Design review of the part shown in the three views and the two pictorial views. Dimensions are in mm from the part's minimum x, y and z. A direction names the side the tool comes from. Coordinates: 2 decimals unless noted, no trailing zeros. Loops run counter-clockwise (first coordinate to the right, second up) from the corner with the lowest first, then second, coordinate; pieces in that order, holes last. Notation, with made-up numbers: (44.25, -26) -> (82.25, -26) arc R6 cw to (82.25, -20) -> close; hole circle Ø8 at (9, 51.25). An arc over 180 degrees is marked (long way). Use CSV: the item, a comma, the result in double quotes.
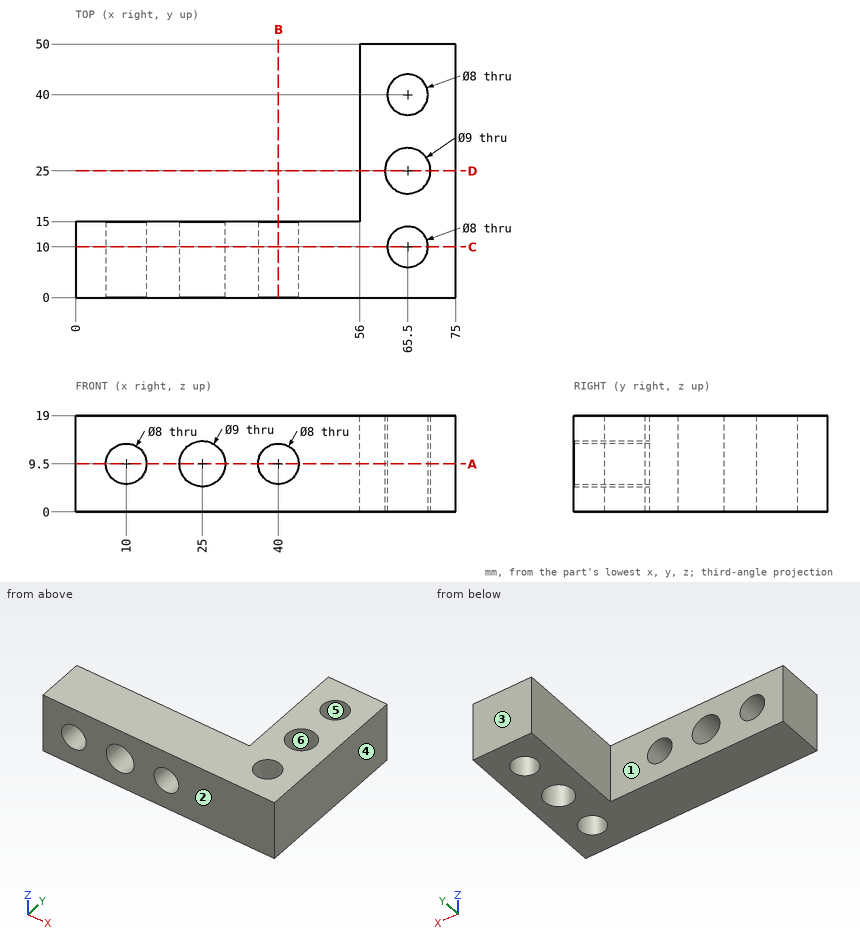
Item 1: Add section D-D (y = 25). Give the boundary of the cut face in (x, z), then the cut area to 3 significant figures.
Checked values:
outline,"(56, 0) -> (61, 0) -> (61, 19) -> (56, 19) -> close; (70, 0) -> (75, 0) -> (75, 19) -> (70, 19) -> close"
area,"190 mm^2"
Item 2: Machinability: for the marked faces 1 and 2, which of the approach directions +Z, -Z, +X, -X, +Y, -Y give a long, thin tool a straight path to every point of the face, cutting with its end or side? Answer none if there is none.
Checked values:
face 1,"+Z, -Z, -X, +Y"
face 2,"+Z, -Z, +X, -X, -Y"
Item 3: Add section C-C (y = 10). Give the boundary of the cut face in (x, z).
Checked values:
outline,"(0, 0) -> (61.5, 0) -> (61.5, 19) -> (0, 19) -> close; (69.5, 0) -> (75, 0) -> (75, 19) -> (69.5, 19) -> close; hole circle Ø8 at (10, 9.5); hole circle Ø9 at (25, 9.5); hole circle Ø8 at (40, 9.5)"
Item 4: Draft analysis for pull direction Y (two halves, no side actions). For the marked faces 3, 4, 5 and 6, state which applies: pulls with the +Y half, pulls with the -Y half, needs draft (parallel to the pull), parting line crosses it, or undercut.
Checked values:
face 3,"pulls with the +Y half"
face 4,"needs draft"
face 5,"undercut"
face 6,"undercut"
Item 5: Clearance check with flat-ended pins moving along their axes: pin 1 (7 mm diameter, centred on x = 65.5, y = 25, fed in from -Z); pin 2 (5.5 mm diameter, centred on y = 39, z = 5, fed in from -X); pin 3 (9.5 mm diameter, centred on x = 23, z = 6.5, fed in from +Y); pin 4 (10.5 mm diameter, centred on x = 65.5, y = 10, fed in from -Z). State where each tip first meets the part, or that it passes through.
Checked values:
pin 1,"through"
pin 2,"x = 56"
pin 3,"y = 15"
pin 4,"z = 0"
Item 6: Add section A-A (z = 9.5). Give the boundary of the cut face in (x, y).
Checked values:
outline,"(0, 0) -> (6, 0) -> (6, 15) -> (0, 15) -> close; (14, 0) -> (20.5, 0) -> (20.5, 15) -> (14, 15) -> close; (29.5, 0) -> (36, 0) -> (36, 15) -> (29.5, 15) -> close; (44, 0) -> (75, 0) -> (75, 50) -> (56, 50) -> (56, 15) -> (44, 15) -> close; hole circle Ø9 at (65.5, 25); hole circle Ø8 at (65.5, 10); hole circle Ø8 at (65.5, 40)"
Item 7: Add section B-B (x = 40). Give the boundary of the cut face in (y, z).
Checked values:
outline,"(0, 0) -> (15, 0) -> (15, 5.5) -> (0, 5.5) -> close; (0, 13.5) -> (15, 13.5) -> (15, 19) -> (0, 19) -> close"
Item 8: To check wall thickness, follow line 1 along Y through (x, z) = (65.5, 9.5); line 2 along Y through (x, z) = (62, 14.25); line 3 along Z through (x, y) = (10, 10.75). State the ranges of each line that lie inside material, in increasing order.
Checked values:
line 1,"0 to 6, 14 to 20.5, 29.5 to 36, 44 to 50"
line 2,"0 to 8.06, 11.94 to 22.17, 27.83 to 38.06, 41.94 to 50"
line 3,"0 to 5.5, 13.5 to 19"
